Verification items for this drawing (mm, ordinates from the low corner). A direction names the side the tool comes from. Give positions to 0.01 mm unless a question says otherwise; leave off trailing zeros. Loops run counter-clockwise (first coordinate to the right, second up) from the corner with the lowest first, then second, coordinate; pieces in that order, holes last. Notation, with made-up numbers: (-23.75, 12) -> (0.25, 12) arc R34 ccw to (0.25, 50) -> close; hole circle Ø9 at (63, 9). An arc over 180 degrees is marked (long way). Write each question's results on one line, items separated by ' | '. Start each with the question number.
Item 1: Cross-section at A-A on y = 16. Enter the section's corners in (x, z).
Item 2: Gauge pin test, flat ends, axial feed: pin 1 Ø4 at (y, z) = (73.5, 89) entering from +X; pin 2 Ø4 at (x, y) = (63, 32.5) entering from +Z; pin 3 Ø3 at (x, y) = (76.5, 15) entering from -Z. Record the tip position at first contact, or that the pin passes through.
Item 3: Cross-section at B-B on y = 79. Enter the section's corners in (x, z).
Item 4: Scan lines: line 1 along X through (y, z) = (53, 77.5); line 2 along X through (y, z) = (68, 77.5); line 3 along Y through (x, z) = (11.5, 56). Record each from-to range of solid material in increasing order.
Item 5: Access from +Z, -Z, +X, -X, +Y, -Y to the whole of each face (thin tool, end or side, straight path). Record for the marked faces 1 and 2.
Item 6: Mould release check, pull along X, two halves, no side actions. Record for the marked faces 3, 4, 5 and 6: pulls with the +X half, pulls with the -X half, needs draft (parallel to the pull), parting line crosses it, or undercut.
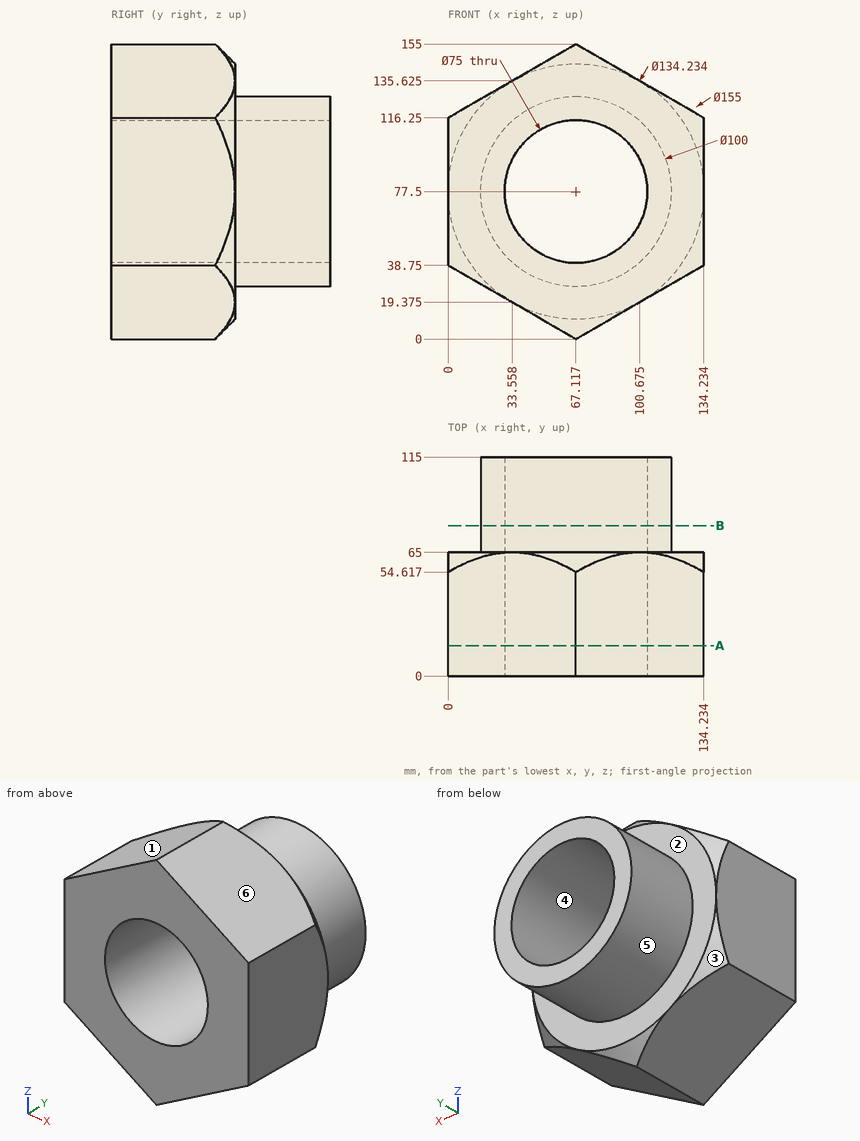
Answer sheet:
1) outline: (0, 38.75) -> (67.12, 0) -> (134.23, 38.75) -> (134.23, 116.25) -> (67.12, 155) -> (0, 116.25) -> close; hole circle Ø75 at (67.12, 77.5)
2) pin 1: stops at x = 116.21 | pin 2: stops at z = 153.78 | pin 3: stops at z = 4.55
3) outline: circle Ø100 at (67.12, 77.5); hole circle Ø75 at (67.12, 77.5)
4) line 1: x = 0 to 29.62, 104.62 to 134.23 | line 2: x = 17.12 to 29.62, 104.62 to 117.12 | line 3: y = 0 to 65
5) face 1: +Z, -X, +Y, -Y | face 2: +Y
6) face 3: pulls with the -X half | face 4: undercut | face 5: parting line crosses it | face 6: pulls with the +X half
